from build123d import *

# Parameters (mm, degrees)
EDGE_CHAMFER_2MM_SIZE = 2
KEYWAY_SKETCH_R       = 4
KEYWAY_CUT_8MM_DEPTH  = 25


with BuildPart() as part:
    # Pulley Profile Sketch → Pulley Body (revolve)
    with BuildSketch(Plane.XY, mode=Mode.PRIVATE) as pulley_body_sk:
        with BuildLine():
            Line((-27.5, 26), (27.5, 26))
            Line((27.5, 26), (27.5, 50))
            Line((27.5, 50), (19, 50))
            Line((19, 50), (19, 80))
            Line((19, 80), (16.25, 80))
            ThreePointArc((16.25, 80), (13.25, 79), (11.45, 76.4))
            Line((11.45, 76.4), (4.8, 53.6))
            ThreePointArc((4.8, 53.6), (0, 50), (-4.8, 53.6))
            Line((-4.8, 53.6), (-11.45, 76.4))
            ThreePointArc((-11.45, 76.4), (-13.25, 79), (-16.25, 80))
            Line((-16.25, 80), (-19, 80))
            Line((-19, 80), (-19, 50))
            Line((-19, 50), (-27.5, 50))
            Line((-27.5, 50), (-27.5, 26))
        make_face()
    revolve(pulley_body_sk.sketch.rotate(Axis((0, 0, 0), (1, 0, 0)), 90), axis=Axis((0, 0, 0), (1, 0, 0)))

    # Edge Chamfer 2mm
    edge_chamfer_2mm_edges = [part.edges().sort_by_distance(p)[0] for p in [
        (27.5, 0, -26),
        (-27.5, 0, -26),
    ]]
    chamfer(edge_chamfer_2mm_edges, length=EDGE_CHAMFER_2MM_SIZE)

    # Keyway Sketch → Keyway Cut 8mm (cut)
    with BuildSketch(Plane(origin=(27.5, 0, 0), x_dir=(0, 0, -1), z_dir=(1, 0, 0))):
        with Locations((0, -26)):
            Circle(KEYWAY_SKETCH_R)
    extrude(amount=-KEYWAY_CUT_8MM_DEPTH, mode=Mode.SUBTRACT)


solid = part.part
Geometry check sheet. Reference: the model listing, model coordinates, mm. A direction names the side the tool comes from. Give positions to 0.01 mm unless a question says otherwise; leave off trailing zeros. Loops run counter-clockwise (first coordinate to the right, second up) from the corner with the lowest first, then second, coordinate; pieces in that order, holes last.
(1) Section check C-C on x = 9. Record the cut outline in (y, z).
From the geometry:
outline: circle Ø136 at (0, 0); hole (-25.69, -3.99) arc R26 ccw (long way) to (-25.69, 3.99) arc R4 ccw (long way) to start
(2) Thickness scan on L1, parallel to X at y = 65, z = -17.5; L2, parallel to X at y = -17, z = 62.5; L3, parallel to Y at x = -3.5, z = 0. Record the ranges inside material, lowest first.
From the geometry:
L1: x = -19 to -8.8, 8.8 to 19
L2: x = -19 to -8.06, 8.06 to 19
L3: y = -51.43 to -26, 26 to 51.43
(3) Depth check by flat-ended pin: pin 1 Ø6 at (x, z) = (21, 11.5) entering from +Y; pin 2 Ø8 at (x, z) = (0, 27.5) entering from -Y; pin 3 Ø1 at (x, z) = (-12, 52) entering from +Y; pin 4 Ø4.5 at (y, z) = (-28.5, -1) entering from +X. Enter the tip coordinate at first touch or a pass-through.
From the geometry:
pin 1: stops at y = 79.46
pin 2: stops at y = -44.63
pin 3: stops at y = 58.67
pin 4: stops at x = 27.5
(4) Set-up check for faces 1 (the conical face through (5.12, 48.53, 25.24)), 2 (the flat face through (-27.5, 22, 22)), 3 (the cylindrical face through (-17.644, -3.517, -79.923)), 4 (the cylindrical face through (15, -30, 0)), 5 (the cylindrical face through (-23.31, -15.02, 47.69)): record each of +Z, -Z, +X, -X, +Y, -Y from which the full face is reachable in a straight line by a thin tool's end or side.
From the geometry:
face 1: none
face 2: +Z, -Z, -X, +Y, -Y
face 3: +X, -X
face 4: +X
face 5: -X
(5) Release check for a two-part mould opening along Z. For faces 6 (the flat face through (2.5, -28, 0)), 7 (the flat face through (27.5, 22, -22)), 8 (the cylindrical face through (23.19, -15.02, 47.69)) record: released by +Z, released by -Z, zero draft, split by the parting line, or undercut.
From the geometry:
face 6: undercut
face 7: zero draft
face 8: split by the parting line
